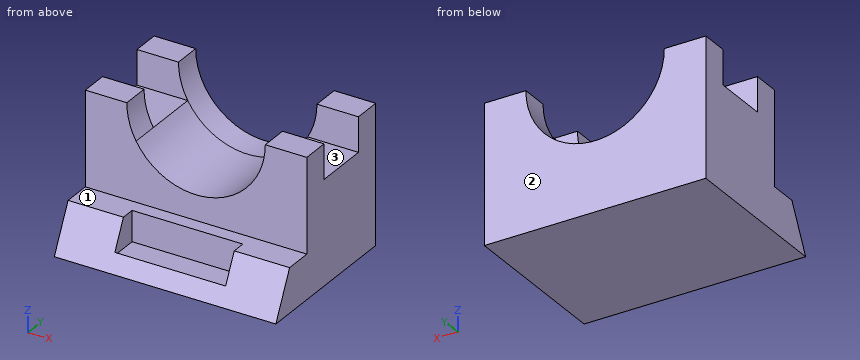
from build123d import *

# Parameters (mm, degrees)
BASE_BLOCK_SKETCH_W        = 80
BASE_BLOCK_SKETCH_H        = 58
BASE_BLOCK_DEPTH           = 16
UPPER_BLOCK_DEPTH          = 10
SIDE_BLOCK_80_DEPTH        = 80
SEMICIRCULAR_BORE_50_DEPTH = 30
RECTANGULAR_SLOT_SKETCH_W  = 43.30127019
RECTANGULAR_SLOT_SKETCH_H  = 12.5
RECTANGULAR_SLOT_DEPTH     = 10
BORE_SIDE_GROOVES_DEPTH    = 10
WEDGE_CUT_DEPTH            = 80
BOTTOM_NOTCH_DEPTH         = 11


with BuildPart() as part:
    # Base Block Sketch → Base Block (new body)
    with BuildSketch(Plane.XY):
        with Locations((40, -29)):
            Rectangle(BASE_BLOCK_SKETCH_W, BASE_BLOCK_SKETCH_H)
    extrude(amount=BASE_BLOCK_DEPTH)

    # Upper Block Sketch → Upper Block (add)
    with BuildSketch(Plane(origin=(0, 0, 0), x_dir=(1, 0, 0), z_dir=(0, 1, 0))):
        with BuildLine():
            Line((0, -16), (0, -50))
            Line((0, -50), (15, -50))
            ThreePointArc((15, -50), (40, -25), (65, -50))
            Line((65, -50), (80, -50))
            Line((80, -50), (80, -16))
            Line((80, -16), (0, -16))
        make_face()
    extrude(amount=-UPPER_BLOCK_DEPTH)

    # Side Block Sketch → Side Block 80 (add)
    with BuildSketch(Plane.ZY):
        Polygon((37.5, -10), (37.5, -30), (50, -30), (50, -40), (16, -40), (16, -10), align=None)
    extrude(amount=-SIDE_BLOCK_80_DEPTH)

    # Bore Ø50 Sketch → Semicircular Bore Ø50 (cut)
    with BuildSketch(Plane(origin=(0, -10, 0), x_dir=(1, 0, 0), z_dir=(0, 1, 0))):
        with BuildLine():
            Line((18.349364905, -37.5), (61.650635095, -37.5))
            ThreePointArc((61.650635095, -37.5), (40, -25), (18.349364905, -37.5))
        make_face()
    extrude(amount=-SEMICIRCULAR_BORE_50_DEPTH, mode=Mode.SUBTRACT)

    # Rectangular Slot Sketch → Rectangular Slot (cut)
    with BuildSketch(Plane.XZ.offset(40)):
        with Locations((40, 43.75)):
            Rectangle(RECTANGULAR_SLOT_SKETCH_W, RECTANGULAR_SLOT_SKETCH_H)
    extrude(amount=-RECTANGULAR_SLOT_DEPTH, mode=Mode.SUBTRACT)

    # Bore Grooves Sketch → Bore Side Grooves (cut)
    with BuildSketch(Plane(origin=(0, -30, 0), x_dir=(1, 0, 0), z_dir=(0, 1, 0))):
        with BuildLine():
            Line((15, -50), (18.349364905, -50))
            Line((18.349364905, -50), (18.349364905, -37.5))
            ThreePointArc((18.349364905, -37.5), (15.851854343, -43.529523872), (15, -50))
        make_face()
        with BuildLine():
            Line((65, -50), (61.650635095, -50))
            Line((61.650635095, -50), (61.650635095, -37.5))
            ThreePointArc((61.650635095, -37.5), (64.148145657, -43.529523872), (65, -50))
        make_face()
    extrude(amount=-BORE_SIDE_GROOVES_DEPTH, mode=Mode.SUBTRACT)

    # Wedge Cut Sketch → Wedge Cut (cut)
    with BuildSketch(Plane.ZY):
        Polygon((16, -50), (0, -58), (16, -58), align=None)
    extrude(amount=-WEDGE_CUT_DEPTH, mode=Mode.SUBTRACT)

    # Bottom Notch Sketch → Bottom Notch (cut)
    with BuildSketch(Plane.XY.offset(16)):
        Polygon((60, -50), (60, -45), (20, -45), (20, -55), (60, -55), align=None)
    extrude(amount=-BOTTOM_NOTCH_DEPTH, mode=Mode.SUBTRACT)


solid = part.part
Source: CAD feature listing. Evaluate the final solid. Frame: model axes, mm. Face numbers are marked on the shaded views. A direction names the side the tool comes from. Coordinates: 2 decimals unless noted, no trailing zeros. Loops run counter-clockwise (first coordinate to the right, second up) from the corner with the lowest first, then second, coordinate; pieces in that order, holes last. Notation, with made-up numbers: (-3.5, -27) - (15.5, -27) arc R32 ccw to (15.5, 8) - close; hole circle Ø7 at (-24, 43.25). An arc over 180 degrees is marked (long way). Return JSON: item names as keys, results as strings.
Q1. Section B-B, the plane z = 39.5. Return loops of the section in (x, y).
Results:
{"outline": "(0, -40) - (17.31, -40) - (17.31, -30) - (0, -30) - close; (0, -10) - (17.31, -10) - (17.31, 0) - (0, 0) - close; (62.69, -40) - (80, -40) - (80, -30) - (62.69, -30) - close; (62.69, -10) - (80, -10) - (80, 0) - (62.69, 0) - close"}
Q2. Section A-A, the plane x = 40. Return loops of the section in (y, z).
Results:
{"outline": "(-58, 0) - (0, 0) - (0, 25) - (-40, 25) - (-40, 16) - (-45, 16) - (-45, 5) - (-55, 5) - (-55, 6) - close"}
Q3. Material intervals for line 1 along Y through (x, z) = (9, 47); line 2 along Y through (x, z) = (66.5, 21); line 3 along X through (y, z) = (-7, 43.5), sorted ascending.
Results:
{"line 1": "-40 to -30, -10 to 0", "line 2": "-40 to 0", "line 3": "0 to 15.86, 64.14 to 80"}
Q4. Access query for the marked faces 1, 2 and 3. Directions: +Z, -Z, +X, -X, +Y, -Y. A direction counts if a zero-diameter tool reaches every point of the face in a straight line with its end or side. Return the directions, or none.
Results:
{"face 1": "+Z, +X, -X, -Y", "face 2": "+Z, -Z, +X, -X, +Y", "face 3": "+Z, +X, -X"}
Q5. Contact query for flat-ended pins moving along their axis: P1, Ø3, axis at x = 44, y = -45.5, coming from the +Z side; P2, Ø2, axis at x = 29.5, z = 22.5, coming from the -Y side; P3, Ø9, axis at x = 69, y = -15.5, coming from the +Z side. Output: stop coordinate, or through.
Results:
{"P1": "z = 16", "P2": "y = -40", "P3": "z = 37.5"}
Q6. Section D-D, the plane z = 10. Return loops of the section in (x, y), plus the area to 3 significant figures.
Results:
{"outline": "(0, -53) - (20, -53) - (20, -45) - (60, -45) - (60, -53) - (80, -53) - (80, 0) - (0, 0) - close", "area": "3,920 mm2"}
Q7. Section C-C, the plane y = -22. Return loops of the section in (x, z).
Results:
{"outline": "(0, 0) - (80, 0) - (80, 37.5) - (61.65, 37.5) arc R25 cw to (18.35, 37.5) - (0, 37.5) - close"}
